```python
from build123d import *

# Parameters (mm, degrees)
SKETCH1_R                  = 17.5
BOSS_EXTRUDE1_DEPTH        = 10
SKETCH2_W                  = 40
SKETCH2_H                  = 19
BOSS_EXTRUDE2_DEPTH        = 10
CHAMFER1_SIZE              = 1
SKETCH3_R                  = 12.5
CUT_EXTRUDE1_DEPTH         = 29.394541729
SKETCH4_W                  = 3
SKETCH4_H                  = 16
CUT_EXTRUDE2_DEPTH         = 29.394541729
M4_TAPPED_HOLE1_D          = 3.3
M4_TAPPED_HOLE1_DEPTH      = 10.1
M4_TAPPED_HOLE1_TIP        = 0.991420021
FILLET1_R                  = 2.5
M3_TAPPED_HOLE1_AT_2_COUNT = 2
M3_TAPPED_HOLE1_AT_2_PITCH = 9
CHAMFER2_SIZE              = 0.5


with BuildPart() as part:
    # Sketch1 → Boss-Extrude1 (new body)
    with BuildSketch(Plane.XY):
        Circle(SKETCH1_R)
    extrude(amount=BOSS_EXTRUDE1_DEPTH)

    # Sketch2 → Boss-Extrude2 (add)
    with BuildSketch(Plane.XY.offset(10)):
        Rectangle(SKETCH2_W, SKETCH2_H)
    extrude(amount=-BOSS_EXTRUDE2_DEPTH)

    # Chamfer1
    chamfer1_edges = [part.edges().sort_by_distance(p)[0] for p in [
        (20, 0, 10),
        (-20, 0, 10),
        (-20, 0, 0),
        (20, 0, 0),
    ]]
    chamfer(chamfer1_edges, length=CHAMFER1_SIZE)

    # Sketch3 → Cut-Extrude1 (cut, through all)
    with BuildSketch(Plane.XY.offset(10)):
        Circle(SKETCH3_R)
    extrude(amount=-CUT_EXTRUDE1_DEPTH, mode=Mode.SUBTRACT)

    # Sketch4 → Cut-Extrude2 (cut, through all)
    with BuildSketch(Plane.XY.offset(10)):
        with Locations((20, 0)):
            Rectangle(SKETCH4_W, SKETCH4_H)
        with Locations((-20, 0)):
            Rectangle(SKETCH4_W, SKETCH4_H)
    extrude(amount=-CUT_EXTRUDE2_DEPTH, mode=Mode.SUBTRACT)

    # M4 Tapped Hole1
    with Locations(Plane.XZ.offset(20.35278131)):
        with Locations((0, 5)):
            Hole(M4_TAPPED_HOLE1_D / 2, depth=M4_TAPPED_HOLE1_DEPTH)
            with Locations((0, 0, -(M4_TAPPED_HOLE1_DEPTH + M4_TAPPED_HOLE1_TIP / 2))):  # 118° drill point
                Cone(0, M4_TAPPED_HOLE1_D / 2, M4_TAPPED_HOLE1_TIP, mode=Mode.SUBTRACT)

    # Fillet1
    fillet1_edges = [part.edges().sort_by_distance(p)[0] for p in [
        (-14.696938457, -9.5, 5),
        (14.696938457, -9.5, 5),
        (14.696938457, 9.5, 5),
        (-14.696938457, 9.5, 5),
    ]]
    fillet(fillet1_edges, radius=FILLET1_R)

    # Sketch7 → M3 Tapped Hole1 (revolve, cut)
    with BuildSketch(Plane(origin=(18.5, -4.5, 5), x_dir=(0, 0, -1), z_dir=(0, 1, 0))):
        Polygon((0, 0), (0, 8.251075774), (1.25, 7.5), (1.25, 0), align=None)
    m3_tapped_hole1 = revolve(axis=Axis((24.85, -4.5, 5), (-1, 0, 0)), mode=Mode.SUBTRACT)

    # M3 Tapped Hole1 at 2: M3 Tapped Hole1 ×2
    with Locations(*[(0, i * M3_TAPPED_HOLE1_AT_2_PITCH, 0) for i in range(1, M3_TAPPED_HOLE1_AT_2_COUNT)]):
        add(m3_tapped_hole1, mode=Mode.SUBTRACT)

    # Mirror1: M3 Tapped Hole1 across plane
    add(m3_tapped_hole1.mirror(Plane(origin=(0, 0, 0), x_dir=(0, 0, 1), z_dir=(1, 0, 0))), mode=Mode.SUBTRACT)

    # Mirror1 copy 1 sketch → Mirror1 copy 1 (revolve, cut)
    with BuildSketch(Plane(origin=(-18.5, 4.5, 5), x_dir=(0, 0, -1), z_dir=(0, 1, 0))):
        Polygon((0, 0), (0, -8.251075774), (1.25, -7.5), (1.25, 0), align=None)
    revolve(axis=Axis((-24.85, 4.5, 5), (-1, 0, 0)), mode=Mode.SUBTRACT)

    # Chamfer2
    chamfer2_edges = [part.edges().sort_by_distance(p)[0] for p in [
        (-12.5, 0, 0),
        (-12.5, 0, 10),
    ]]
    chamfer(chamfer2_edges, length=CHAMFER2_SIZE)


solid = part.part
```
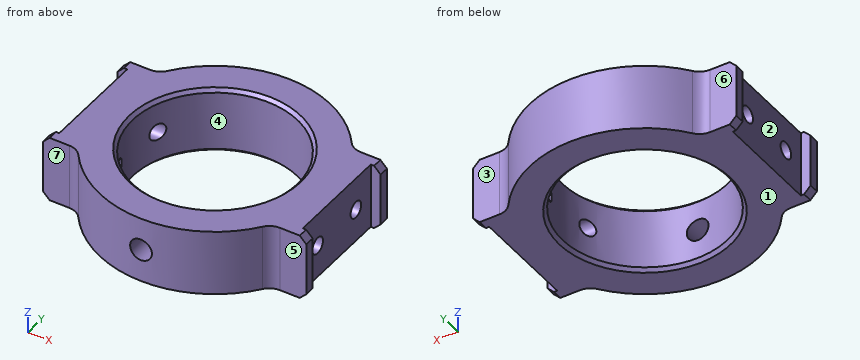
Can you work these out from the model? Positions are in its coordinate system, mm. Face numbers are marked on the shaded views. A direction names the side the tool comes from. Round coordinates to 2 decimals unless told otherwise and drop trailing zeros. Order: outer loops, then holes, each group sorted by start corner. A loop starts at its lowest first (then second) coordinate and runs counter-clockwise, first axis right, second up.
(1) If we section it at C-C (x = 15): Please give me the cut outline in (y, z).
Results are:
outline: (-9.71, 0) - (9.71, 0) - (9.71, 10) - (-9.71, 10) - close; hole circle Ø2.5 at (-4.5, 5); hole circle Ø2.5 at (4.5, 5)
(2) I'm going to push flat-ended pins straight in: pin 1 (2 mm diameter, centred on x = 17, z = 6, fed in from +Y); pin 2 (1.6 mm diameter, centred on x = -19, z = 7.5, fed in from -Y); pin 3 (1 mm diameter, centred on y = -4.5, z = 6.5, fed in from +X). Where does each tip first touch, or does it pass through?
Results are:
pin 1: stops at y = 9.5
pin 2: stops at y = -9.5
pin 3: stops at x = 18.5
(3) If we section it at A-A (x = 0): Please give me the cut outline in (y, z).
Results are:
outline: (-17.5, 0) - (-13, 0) - (-12.5, 0.5) - (-12.5, 3.35) - (-17.5, 3.35) - close; (-17.5, 6.65) - (-12.5, 6.65) - (-12.5, 9.5) - (-13, 10) - (-17.5, 10) - close; (12.5, 0.5) - (13, 0) - (17.5, 0) - (17.5, 10) - (13, 10) - (12.5, 9.5) - close
(4) If we section it at D-D (z = 5): Count the separate pieces of the cut face and the enclosed holes in it, plus the area to 3 significant figures.
Results are:
separate pieces: 5
enclosed holes: 0
area: 468 mm2
(5) If I drill on L1, parallel to Z at x = 15, y = -4.5; L2, parallel to Y at x = 17.5, z = 6; L3, parallel to Y at x = -16, z = 9, over which ranges is the centre line in solid material (lowest first)?
Results are:
L1: z = 0 to 3.75, 6.25 to 10
L2: y = -9.5 to -5.25, -3.75 to 3.75, 5.25 to 9.5
L3: y = -9.5 to 9.5
(6) On a 3-axis mill with a long thin cutter (end or side, diameter ignored), from which of +Z, -Z, +X, -X, +Y, -Y can I reach the whole of each face in a straight line? I mean the marked faces 5, 6 and 7. Say none if no direction works.
Results are:
face 5: +Z, -Z, +X, -Y
face 6: +Z, -Z, -X, +Y
face 7: +Z, -Z, -X, -Y
(7) If we section it at B-B (y = 0): Please give me the cut outline in (x, z).
Results are:
outline: (-18.5, 0) - (-13, 0) - (-12.5, 0.5) - (-12.5, 9.5) - (-13, 10) - (-18.5, 10) - close; (12.5, 0.5) - (13, 0) - (18.5, 0) - (18.5, 10) - (13, 10) - (12.5, 9.5) - close
(8) We'd pull the mould along Y, two halves only. Please class the marked faces 1, 2, 3 and 4: +Y half, -Y half, draft (parallel to the pull), parting line (faces both ways), or undercut.
Results are:
face 1: draft
face 2: undercut
face 3: +Y half
face 4: undercut
